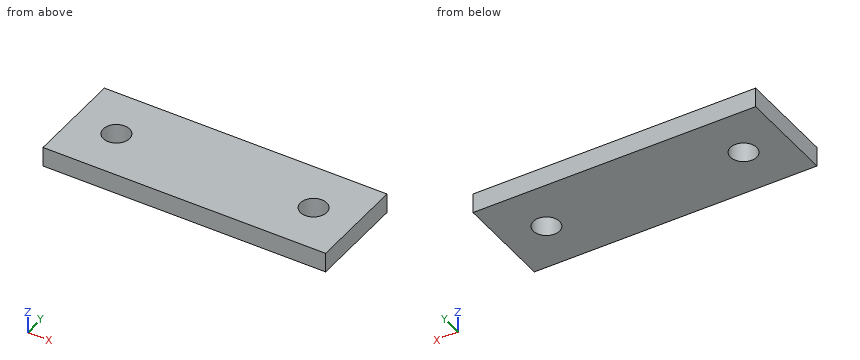
```python
from build123d import *

# Parameters (mm, degrees)
SKETCH1_W           = 86
SKETCH1_H           = 30
BOSS_EXTRUDE1_DEPTH = 6
SKETCH2_R           = 4
CUT_EXTRUDE1_DEPTH  = 10


with BuildPart() as part:
    # Sketch1 → Boss-Extrude1 (new body)
    with BuildSketch(Plane.XY):
        Rectangle(SKETCH1_W, SKETCH1_H)
    extrude(amount=BOSS_EXTRUDE1_DEPTH)

    # Sketch2 → Cut-Extrude1 (cut)
    with BuildSketch(Plane.XY.offset(6)):
        with Locations((-30, 0)):
            Circle(SKETCH2_R)
        with Locations((30, 0)):
            Circle(SKETCH2_R)
    extrude(amount=-CUT_EXTRUDE1_DEPTH, mode=Mode.SUBTRACT)


solid = part.part
```
Here's how the part is built. I have some questions about the finished solid (model axes, mm). Round coordinates to 2 decimals unless told otherwise and drop trailing zeros. Write each loop counter-clockwise with the first axis right and the second up, starting at its lowest first coordinate (ties: lowest second). Pieces come first, ordered by that corner, then holes.
Q1. If we section it at D-D on x = -31: Write out the boundary of the cut face in (y, z), plus the area to 3 significant figures.
Q2. If we section it at C-C on z = 1.7: Write out the boundary of the cut face in (x, y), plus the area to 3 significant figures.
Q3. If we section it at B-B on x = 30: Write out the boundary of the cut face in (y, z).
Q4. Please list where these lines run through material, in increasing order: probe 1 along Y at (x, z) = (30, 4.2); probe 2 along X at (y, z) = (-2, 5.3); probe 3 along Y at (x, z) = (-26.5, 0.9).
Q5. If we section it at A-A on y = 0: Write out the boundary of the cut face in (x, z).
Answer below:
1. outline: (-15, 0) - (-3.87, 0) - (-3.87, 6) - (-15, 6) - close; (3.87, 0) - (15, 0) - (15, 6) - (3.87, 6) - close
1. area: 134 mm2
2. outline: (-43, -15) - (43, -15) - (43, 15) - (-43, 15) - close; hole circle Ø8 at (-30, 0); hole circle Ø8 at (30, 0)
2. area: 2,480 mm2
3. outline: (-15, 0) - (-4, 0) - (-4, 6) - (-15, 6) - close; (4, 0) - (15, 0) - (15, 6) - (4, 6) - close
4. probe 1: y = -15 to -4, 4 to 15
4. probe 2: x = -43 to -33.46, -26.54 to 26.54, 33.46 to 43
4. probe 3: y = -15 to -1.94, 1.94 to 15
5. outline: (-43, 0) - (-34, 0) - (-34, 6) - (-43, 6) - close; (-26, 0) - (26, 0) - (26, 6) - (-26, 6) - close; (34, 0) - (43, 0) - (43, 6) - (34, 6) - close
